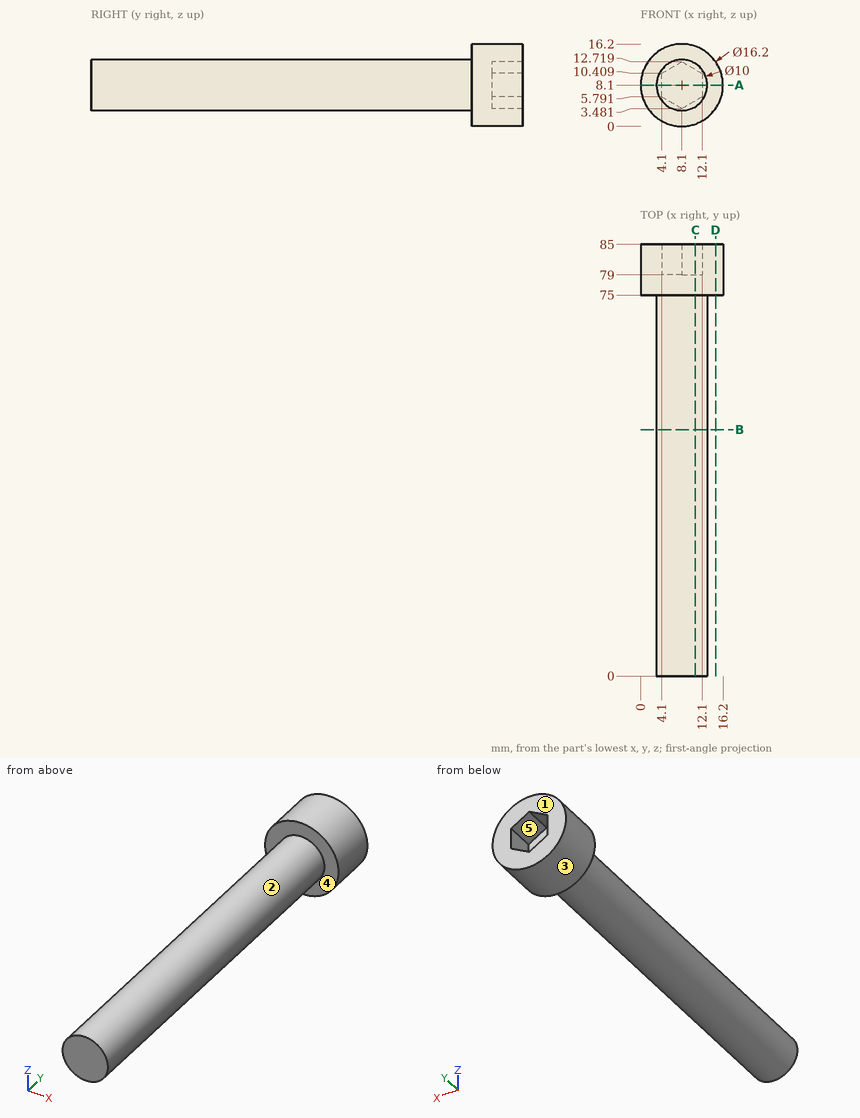
Input: dimensioned drawing with shaded views. Units: mm. Origin: part minimum x, y, z. A direction names the side the tool comes from. Round coordinates to 2 decimals unless told otherwise and drop trailing zeros. Order: outer loops, then holes, each group sorted by start corner. A loop starts at its lowest first (then second) coordinate and runs counter-clockwise, first axis right, second up. Notation, with made-up numbers: (-15, 44.5) - (1, 44.5) arc R20 cw to (1, 49.5) - close; hole circle Ø10 at (50.5, 29). An arc over 180 degrees is marked (long way). Use CSV: the item, a comma, the result in double quotes. Start each with the question number.
Q1. Section query B-B (y = 48.5). Return loops of the section in (x, z).
Q2. Section query A-A (z = 8.1). Return loops of the section in (x, y), and give its area (3 significant figures).
Q3. Mould query, pull axis Z, two halves, no side actions, for the marked faces 3, 4 and 5. Classes: +Z half, -Z half, draft (parallel to the pull), parting line (faces both ways), or undercut.
Q4. Section query C-C (x = 10.75). Return loops of the section in (y, z) (1 decimal), and give its area (3 significant figures).
Q5. Material intervals for line 1 along Y through (x, z) = (14, 10.25); line 2 along Y through (x, z) = (4.75, 9.75); line 3 along X through (y, z) = (5, 8.25), sorted ascending. Write a range as from..to.
Q6. Section query D-D (x = 14.75). Return loops of the section in (y, z) (1 decimal), and give its area (3 significant figures).
Q7. First-contact query: pin 1 (6 mm diameter, centred on x = 13, y = 74.5, fed in from -Z); pin 2 (1 mm diameter, centred on y = 37, z = 3.5, fed in from +X); pin 3 (6 mm diameter, centred on y = 13.5, z = 7.5, fed in from -X). Flat tips, straight axial feed; report the tip coordinate or a pass-through.
Q8. Access query for the marked faces 1 and 2. Directions: +Z, -Z, +X, -X, +Y, -Y. A direction counts if a zero-diameter tool reaches every point of the face in a straight line with its end or side. Return the directions, or none.
Result set:
1,outline,"circle Ø10 at (8.1, 8.1)"
2,outline,"(0, 75) - (3.1, 75) - (3.1, 0) - (13.1, 0) - (13.1, 75) - (16.2, 75) - (16.2, 85) - (12.1, 85) - (12.1, 79) - (4.1, 79) - (4.1, 85) - (0, 85) - close"
2,area,"864 mm2"
3,face 3,"parting line"
3,face 4,"draft"
3,face 5,"undercut"
4,outline,"(0, 3.9) - (75, 3.9) - (75, 0.4) - (85, 0.4) - (85, 5) - (79, 5) - (79, 11.2) - (85, 11.2) - (85, 15.8) - (75, 15.8) - (75, 12.3) - (0, 12.3) - close"
4,area,"752 mm2"
5,line 1,"y = 75..85"
5,line 2,"y = 0..79"
5,line 3,"x = 3.1..13.1"
6,outline,"(75, 3.5) - (85, 3.5) - (85, 12.7) - (75, 12.7) - close"
6,area,"92.5 mm2"
7,pin 1,"stops at z = 0.24"
7,pin 2,"stops at x = 10.96"
7,pin 3,"stops at x = 3.1"
8,face 1,"+Z, -Z, +X, -X, +Y"
8,face 2,"-Y"
